Geometry check sheet. Reference: the model listing, model coordinates, mm. Face numbers are marked on the shaded views. A direction names the side the tool comes from. Coordinates: 2 decimals unless noted, no trailing zeros. Order: outer loops, then holes, each group sorted by start corner. A loop starts at its lowest first (then second) coordinate and runs counter-clockwise, first axis right, second up. Notation, with made-up numbers: (81.25, 38) -> (131.25, 38) arc R7 ccw to (131.25, 46) -> close; hole circle Ø5 at (50.25, 1). An arc over 180 degrees is marked (long way). Answer in a Markdown table with one row per item. Add a question column.
```python
from build123d import *

# Parameters (mm, degrees)
SKETCH1_R           = 7.5
BOSS_EXTRUDE1_DEPTH = 15
SKETCH2_R           = 4
BOSS_EXTRUDE2_DEPTH = 10
CHAMFER1_SIZE       = 0.5


with BuildPart() as part:
    # Sketch1 → Boss-Extrude1 (new body)
    with BuildSketch(Plane.XY):
        Circle(SKETCH1_R)
    extrude(amount=BOSS_EXTRUDE1_DEPTH)

    # Sketch2 → Boss-Extrude2 (add)
    with BuildSketch(Plane.XY.offset(15)):
        Circle(SKETCH2_R)
    extrude(amount=BOSS_EXTRUDE2_DEPTH)

    # Chamfer1
    chamfer1_edges = [part.edges().sort_by_distance(p)[0] for p in [
        (-7.5, 0, 0),
        (-7.5, 0, 15),
        (-4, 0, 25),
    ]]
    chamfer(chamfer1_edges, length=CHAMFER1_SIZE)


solid = part.part
```
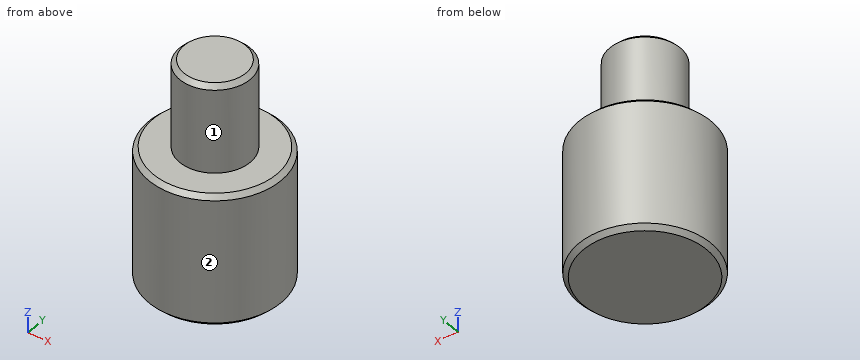
(1) Scan lines: line 1 along Z through (x, y) = (-2, -3.75); line 2 along Y through (x, z) = (-0.25, 2.5); line 3 along Y through (x, z) = (-2.25, 19.75). Record each from-to range of solid material in increasing order.
(2) Cross-section at C-C (z = 19.5). Enter the section's corners in (x, y), plus the area to 3 significant figures.
(3) Cross-section at D-D (z = 13). Enter the section's corners in (x, y).
(4) Cross-section at A-A (y = 0). Enter the section's corners in (x, z).
(5) Go/stop test with flat-tipped pins: P1, Ø1.5, axis at x = 5, y = 2.5, coming from the -Z side; P2, Ø1, axis at y = -0.5, z = 16.5, coming from the +X side; P3, Ø3, axis at x = 6, z = 13.5, coming from the +Y side; P4, Ø6, axis at x = 5, y = 4.5, coming from the +Z side. Record where each tip stops, or that it passes through.
(6) Access from +Z, -Z, +X, -X, +Y, -Y to the whole of each face (thin tool, end or side, straight path). Record for the marked faces 1 and 2.
Checks:
| question | item | result |
|---|---|---|
| 1 | line 1 | 0 to 15 |
| 1 | line 2 | -7.5 to 7.5 |
| 1 | line 3 | -3.31 to 3.31 |
| 2 | outline | circle Ø8 at (0, 0) |
| 2 | area | 50.3 mm² |
| 3 | outline | circle Ø15 at (0, 0) |
| 4 | outline | (-7.5, 0.5) -> (-7, 0) -> (7, 0) -> (7.5, 0.5) -> (7.5, 14.5) -> (7, 15) -> (4, 15) -> (4, 24.5) -> (3.5, 25) -> (-3.5, 25) -> (-4, 24.5) -> (-4, 15) -> (-7, 15) -> (-7.5, 14.5) -> close |
| 5 | P1 | z = 0 |
| 5 | P2 | x = 4 |
| 5 | P3 | y = 6 |
| 5 | P4 | z = 24.77 |
| 6 | face 1 | +Z |
| 6 | face 2 | +Z, -Z |
